Build history of the part. All positions in model axes, mm. A direction names the side the tool comes from. Round coordinates to 2 decimals unless told otherwise and drop trailing zeros. Loops run counter-clockwise (first coordinate to the right, second up) from the corner with the lowest first, then second, coordinate; pieces in that order, holes last. Notation, with made-up numbers: (-3.5, 8) - (21.5, 8) arc R23 cw to (21.5, 22) - close; hole circle Ø8 at (52.5, 75). An arc over 180 degrees is marked (long way). Use a Markdown table: item, result.
from build123d import *

# Parameters (mm, degrees)
SKETCH_1_W             = 85
SKETCH_1_H             = 85
EXTRUDE_1_DEPTH        = 6
SKETCH_2_R             = 25
EXTRUDE_2_DEPTH        = 1
SKETCH_3_R             = 22
CUT_EXTRUDE_1_DEPTH    = 62.493902137
SKETCH_4_R             = 35
CUT_EXTRUDE_2_DEPTH    = 4
HOLE_WIZARD_M6_1_D     = 5
CHAMFER_1_SIZE         = 5
PZ_000000C_D           = 4.5
PZ_000000C_CBORE_D     = 8
PZ_000000C_CBORE_DEPTH = 9


with BuildPart() as part:
    # 草图1 → 凸台-拉伸1 (new, symmetric)
    with BuildSketch(Plane(origin=(0, 0, 0), x_dir=(1, 0, 0), z_dir=(0, 1, 0))):
        Rectangle(SKETCH_1_W, SKETCH_1_H)
    extrude(amount=EXTRUDE_1_DEPTH, both=True)

    # 草图2 → 凸台-拉伸2 (add, symmetric)
    with BuildSketch(Plane.XZ.offset(6)):
        with Locations(Location((0, 0, 0), (0, 0, 270))):
            Circle(SKETCH_2_R)
    extrude(amount=EXTRUDE_2_DEPTH, both=True)

    # 草图3 → 切除-拉伸1 (cut, through all)
    with BuildSketch(Plane.XZ.offset(7)):
        with Locations(Location((0, 0, 0), (0, 0, 270))):
            Circle(SKETCH_3_R)
    extrude(amount=-CUT_EXTRUDE_1_DEPTH, mode=Mode.SUBTRACT)

    # 草图4 → 切除-拉伸2 (cut)
    with BuildSketch(Plane(origin=(0, 6, 0), x_dir=(1, 0, 0), z_dir=(0, 1, 0))):
        with Locations(Location((0, 0, 0), (0, 0, 270))):
            Circle(SKETCH_4_R)
    extrude(amount=-CUT_EXTRUDE_2_DEPTH, mode=Mode.SUBTRACT)

    # M6 螺纹孔1 (through all)
    with Locations(Plane(origin=(0, 6, 0), x_dir=(1, 0, 0), z_dir=(0, 1, 0))):
        with Locations((-31.75, 31.75), (0, 0), (31.75, -31.75), (31.75, 31.75), (-31.75, -31.75)):
            Hole(HOLE_WIZARD_M6_1_D / 2)

    # 倒角1
    chamfer_1_edges = [part.edges().sort_by_distance(p)[0] for p in [
        (42.5, 0, 42.5),
        (-42.5, 0, 42.5),
        (-42.5, 0, -42.5),
        (42.5, 0, -42.5),
    ]]
    chamfer(chamfer_1_edges, length=CHAMFER_1_SIZE)

    # PZ-000000C 铺砖车 (through all)
    with Locations(Plane(origin=(0, 6, 0), x_dir=(1, 0, 0), z_dir=(0, 1, 0))):
        with Locations((-24.748737342, 24.748737341), (24.748737342, 24.748737342), (24.748737342, -24.748737342), (-24.748737342, -24.748737342)):
            CounterBoreHole(PZ_000000C_D / 2, PZ_000000C_CBORE_D / 2, PZ_000000C_CBORE_DEPTH)


solid = part.part
Q1. Cut at C-C, the plane x = -31.75. List the corners of the cut face in (y, z), plus the area to 3 significant figures.
Results found:
| item | result |
|---|---|
| outline | (-6, -42.5) - (6, -42.5) - (6, -34.25) - (-6, -34.25) - close; (-6, -29.25) - (6, -29.25) - (6, -14.73) - (2, -14.73) - (2, 14.73) - (6, 14.73) - (6, 29.25) - (-6, 29.25) - close; (-6, 34.25) - (6, 34.25) - (6, 42.5) - (-6, 42.5) - close |
| area | 782 mm2 |
Q2. Probe line 1 (Z direction, x = 0.5, y = 2.5); line 2 (Z direction, x = 31.75, y = -0.5); line 3 (Z direction, x = -26.5, y = 1.5) (3 decimals). List the from-to ranges inside material, lowest first.
Results found:
| item | result |
|---|---|
| line 1 | z = -42.5 to -35, 35 to 42.5 |
| line 2 | z = -42.5 to -34.25, -29.25 to 29.25, 34.25 to 42.5 |
| line 3 | z = -42.5 to -28.345, -21.152 to 21.152, 28.345 to 42.5 |
Q3. Which spindle directions (+Z, -Z, +X, -X, +Y, -Y) get a long thin tool onto all of the face, cutting with end or side? Do faces 1 (the face through (28.444, 0.563, 26.281)), 2 (the face through (40, 0, 40)). Say none if no direction does.
Results found:
| item | result |
|---|---|
| face 1 | +Y |
| face 2 | +Z, +X, +Y, -Y |
Q4. Cut at A-A, the plane z = 0. List the corners of the cut face in (x, y).
Results found:
| item | result |
|---|---|
| outline | (-42.5, -6) - (-25, -6) - (-25, -7) - (-22, -7) - (-22, 2) - (-35, 2) - (-35, 6) - (-42.5, 6) - close; (22, -7) - (25, -7) - (25, -6) - (42.5, -6) - (42.5, 6) - (35, 6) - (35, 2) - (22, 2) - close |
Q5. Cut at B-B, the plane x = 0. List the corners of the cut face in (y, z).
Results found:
| item | result |
|---|---|
| outline | (-7, -25) - (-6, -25) - (-6, -42.5) - (6, -42.5) - (6, -35) - (2, -35) - (2, -22) - (-7, -22) - close; (-7, 22) - (2, 22) - (2, 35) - (6, 35) - (6, 42.5) - (-6, 42.5) - (-6, 25) - (-7, 25) - close |
Q6. Pull direction X, two halves, no side cores. Call faces 3 (the face through (7.509, -6.507, -23.846)), 4 (the face through (42.5, 0, 1)), 5 (the face through (-22.5, -4.52, 24.65)): pulls with the +X half, pulls with the -X half, needs draft (parallel to the pull), parting line crosses it, or undercut.
Results found:
| item | result |
|---|---|
| face 3 | parting line crosses it |
| face 4 | pulls with the +X half |
| face 5 | undercut |
Q7. Drop flat-ended pins along their axis: pin 1 (5 mm diameter, centred on x = 24.75, z = -24.75, fed in from +Y); pin 2 (4 mm diameter, centred on x = 0.5, z = -21, fed in from +Y); pin 3 (8 mm diameter, centred on x = 29.5, z = -33, fed in from -Y). Give the stop position or say it passes through.
Results found:
| item | result |
|---|---|
| pin 1 | stops at y = -3 |
| pin 2 | stops at y = 2 |
| pin 3 | stops at y = -6 |
Q8. Cut at D-D, the plane z = 31.75. List the corners of the cut face in (x, y).
Results found:
| item | result |
|---|---|
| outline | (-42.5, -6) - (-34.25, -6) - (-34.25, 6) - (-42.5, 6) - close; (-29.25, -6) - (29.25, -6) - (29.25, 6) - (14.73, 6) - (14.73, 2) - (-14.73, 2) - (-14.73, 6) - (-29.25, 6) - close; (34.25, -6) - (42.5, -6) - (42.5, 6) - (34.25, 6) - close |
